Source: CAD feature listing. Evaluate the final solid. Frame: model axes, mm. Round coordinates to 2 decimals unless told otherwise and drop trailing zeros. Order: outer loops, then holes, each group sorted by start corner. A loop starts at its lowest first (then second) coordinate and runs counter-clockwise, first axis right, second up.
```python
from build123d import *

# Parameters (mm, degrees)
SKETCH_1_W                     = 270
SKETCH_1_H                     = 255
EXTRUDE_1_DEPTH                = 6
SKETCH_2_W                     = 95
SKETCH_2_H                     = 95
CUT_EXTRUDE_1_DEPTH            = 12
HOLE_WIZARD_M8_1_D             = 6.8
HOLE_WIZARD_M8_2_D             = 6.8
CHAMFER_1_SIZE                 = 5
CHAMFER_2_SIZE                 = 2
HOLE_WIZARD_M8_2_2_D           = 9
HOLE_WIZARD_M8_2_2_CBORE_D     = 15
HOLE_WIZARD_M8_2_2_CBORE_DEPTH = 8.6
FILLET_1_R                     = 10
HOLE_WIZARD_M5_3_AT_2_COUNT    = 2
HOLE_WIZARD_M5_3_AT_2_PITCH    = 50
HOLE_WIZARD_M5_4_D             = 4.2


with BuildPart() as part:
    # 草图1 → 凸台-拉伸1 (new, symmetric)
    with BuildSketch(Plane.XY):
        Rectangle(SKETCH_1_W, SKETCH_1_H)
    extrude(amount=EXTRUDE_1_DEPTH, both=True)

    # 草图2 → 切除-拉伸1 (cut)
    with BuildSketch(Plane(origin=(0, 0, -6), x_dir=(-1, 0, 0), z_dir=(0, 0, -1))):
        with Locations((87.5, 80)):
            Rectangle(SKETCH_2_W, SKETCH_2_H)
        with Locations((-87.5, 80)):
            Rectangle(SKETCH_2_W, SKETCH_2_H)
    extrude(amount=-CUT_EXTRUDE_1_DEPTH, mode=Mode.SUBTRACT)

    # Hole Wizard M8 _1 (through all)
    with Locations(Plane(origin=(0, 0, -6), x_dir=(-1, 0, 0), z_dir=(0, 0, -1))):
        with Locations((-25, 118.5), (25, 118.5)):
            Hole(HOLE_WIZARD_M8_1_D / 2)

    # Hole Wizard M8 _2 (through all)
    with Locations(Plane(origin=(0, 0, -6), x_dir=(-1, 0, 0), z_dir=(0, 0, -1))):
        with Locations((-45, -92.5), (45, -92.5), (-45, 17.5), (45, 17.5), (-103, 11), (103, 11)):
            Hole(HOLE_WIZARD_M8_2_D / 2)

    # 倒角1
    chamfer_1_edges = [part.edges().sort_by_distance(p)[0] for p in [
        (-40, 127.5, 0),
        (40, 127.5, 0),
    ]]
    chamfer(chamfer_1_edges, length=CHAMFER_1_SIZE)

    # 倒角2
    chamfer_2_edges = [part.edges().sort_by_distance(p)[0] for p in [
        (-135, 32.5, 0),
        (135, 32.5, 0),
        (135, -127.5, 0),
        (-135, -127.5, 0),
    ]]
    chamfer(chamfer_2_edges, length=CHAMFER_2_SIZE)

    # Hole Wizard M8 _2 2 (through all)
    with Locations(Plane.XY.offset(6)):
        with Locations((-50, -25), (-50, -75), (0, -25), (0, -75), (50, -25), (50, -75)):
            CounterBoreHole(HOLE_WIZARD_M8_2_2_D / 2, HOLE_WIZARD_M8_2_2_CBORE_D / 2, HOLE_WIZARD_M8_2_2_CBORE_DEPTH)

    # 圆角1
    fillet_1_edges = [part.edges().sort_by_distance(p)[0] for p in [
        (-40, 32.5, 0),
        (40, 32.5, 0),
    ]]
    fillet(fillet_1_edges, radius=FILLET_1_R)

    # 草图24 → M5 螺纹孔3 (revolve, cut)
    with BuildSketch(Plane(origin=(-135, -75, 0), x_dir=(0, 0, 1), z_dir=(0, 1, 0))):
        Polygon((0, 0), (0, 13.6618073), (2.1, 12.4), (2.1, 0), align=None)
    hole_wizard_m5_3 = revolve(axis=Axis((-141.35, -75, 0), (1, 0, 0)), mode=Mode.SUBTRACT)

    # M5 螺纹孔3 at 2: M5 螺纹孔3 ×2
    with Locations(*[(0, i * HOLE_WIZARD_M5_3_AT_2_PITCH, 0) for i in range(1, HOLE_WIZARD_M5_3_AT_2_COUNT)]):
        add(hole_wizard_m5_3, mode=Mode.SUBTRACT)

    # 镜向1: M5 螺纹孔3 across plane
    add(hole_wizard_m5_3.mirror(Plane.ZY), mode=Mode.SUBTRACT)

    # 镜向1 copy 1 sketch → 镜向1 copy 1 (revolve, cut)
    with BuildSketch(Plane(origin=(135, -25, 0), x_dir=(0, 0, 1), z_dir=(0, 1, 0))):
        Polygon((0, 0), (0, -13.6618073), (2.1, -12.4), (2.1, 0), align=None)
    revolve(axis=Axis((141.35, -25, 0), (1, 0, 0)), mode=Mode.SUBTRACT)

    # M5 螺纹孔4 (through all)
    with Locations(Plane.XY.offset(6)):
        with Locations((0, -121.5)):
            Hole(HOLE_WIZARD_M5_4_D / 2)


solid = part.part
```
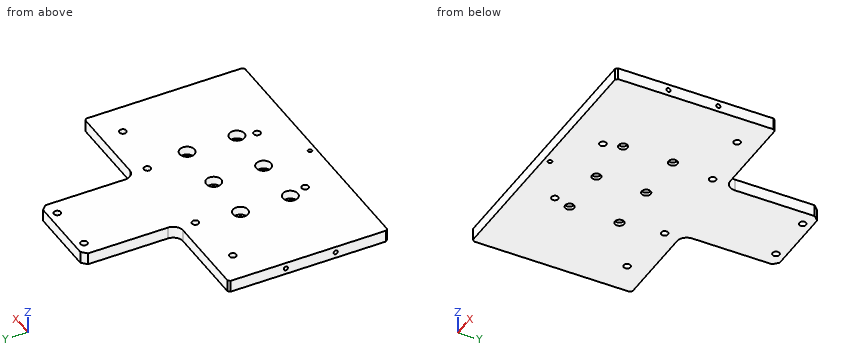
1. Section D-D on y = -92.5. Return loops of the section in (x, z).
2. Section A-A on x = -103. Return loops of the section in (y, z).
3. Line query: line 1 along Y through (x, z) = (-132, 0); line 2 along X through (y, z) = (-19, 2.25); line 3 along Y through (x, z) = (-50, 4.25). Output: solid intervals per line, ascending.
4. Section C-C on x = -25. Return loops of the section in (y, z).
5. First-contact query: pin 1 (4 mm diameter, centred on y = 88, z = -4, fed in from -X); pin 2 (2.5 mm diameter, centred on y = -75, z = 0, fed in from -X); pin 3 (4.5 mm diameter, centred on x = 51.5, y = -77, fed in from +Z). Flat tips, straight axial feed; report the tip coordinate or a pass-through.
6. Section B-B on y = 118.5. Return loops of the section in (x, z), plus the area to 3 significant figures.
Result:
1. outline: (-135, -6) - (-48.4, -6) - (-48.4, 6) - (-135, 6) - close; (-41.6, -6) - (41.6, -6) - (41.6, 6) - (-41.6, 6) - close; (48.4, -6) - (135, -6) - (135, 6) - (48.4, 6) - close
2. outline: (-127.5, -6) - (7.6, -6) - (7.6, 6) - (-127.5, 6) - close; (14.4, -6) - (32.5, -6) - (32.5, 6) - (14.4, 6) - close
3. line 1: y = -127.5 to -77.1, -72.9 to -27.1, -22.9 to 32.5
3. line 2: x = -135 to -54.5, -45.5 to -4.5, 4.5 to 45.5, 54.5 to 135
3. line 3: y = -127.5 to -82.5, -67.5 to -32.5, -17.5 to 32.5
4. outline: (-127.5, -6) - (115.1, -6) - (115.1, 6) - (-127.5, 6) - close; (121.9, -6) - (127.5, -6) - (127.5, 6) - (121.9, 6) - close
5. pin 1: stops at x = -40
5. pin 2: stops at x = -122.09
5. pin 3: stops at z = -2.6
6. outline: (-40, -6) - (-28.4, -6) - (-28.4, 6) - (-40, 6) - close; (-21.6, -6) - (21.6, -6) - (21.6, 6) - (-21.6, 6) - close; (28.4, -6) - (40, -6) - (40, 6) - (28.4, 6) - close
6. area: 797 mm2
